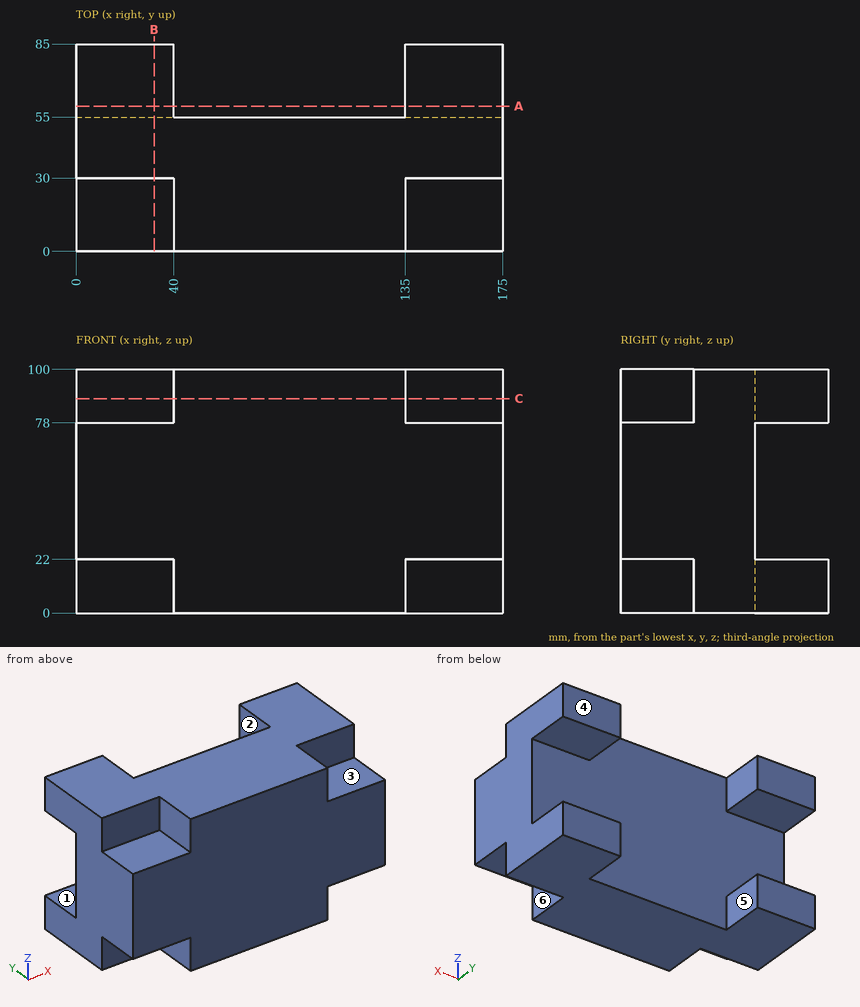
Verification items for this drawing (mm, ordinates from the low corner). A direction names the side the tool comes from. Give positions to 0.01 mm unless a question says otherwise; leave off trailing zeros. Loops run counter-clockwise (first coordinate to the right, second up) from the corner with the lowest first, then second, coordinate; pieces in that order, holes last.
1. Cross-section at C-C on z = 88. Record the cut outline in (x, y), and give its area (4 significant figures).
Derived:
outline: (0, 30) - (40, 30) - (40, 0) - (135, 0) - (135, 30) - (175, 30) - (175, 85) - (135, 85) - (135, 55) - (40, 55) - (40, 85) - (0, 85) - close
area: 9,625 mm2
2. Go/stop test with flat-tipped pins: P1, Ø17.5, axis at y = 17, z = 90.5, coming from the +X side; P2, Ø9, axis at x = 154, y = 12, coming from the +Z side; P3, Ø11, axis at x = 25.5, z = 90, coming from the -Y side. Record where each tip stops, or that it passes through.
Derived:
P1: stops at x = 135
P2: stops at z = 78
P3: stops at y = 30
3. Material ranges on probe 1 along Z at (x, y) = (140, 68.5); probe 2 along X at (y, z) = (58, 81.5); probe 3 along Y at (x, z) = (75, 18.5), recorded low to high.
Derived:
probe 1: z = 0 to 22, 78 to 100
probe 2: x = 0 to 40, 135 to 175
probe 3: y = 0 to 55
4. Cross-section at A-A on y = 59.5. Record the cut outline in (x, z).
Derived:
outline: (0, 0) - (40, 0) - (40, 22) - (0, 22) - close; (0, 78) - (40, 78) - (40, 100) - (0, 100) - close; (135, 0) - (175, 0) - (175, 22) - (135, 22) - close; (135, 78) - (175, 78) - (175, 100) - (135, 100) - close
5. Release check for a two-part mould opening along X. For the marked faces 4, 5 and 6 record: +X half, -X half, draft (parallel to the pull), parting line (faces both ways), or undercut.
Derived:
face 4: draft
face 5: undercut
face 6: +X half
6. Cross-section at B-B on x = 32. Record the cut outline in (y, z), and give its area (3 significant figures).
Derived:
outline: (0, 22) - (30, 22) - (30, 0) - (85, 0) - (85, 22) - (55, 22) - (55, 78) - (85, 78) - (85, 100) - (30, 100) - (30, 78) - (0, 78) - close
area: 5,500 mm2
7. Tool access check on the marked faces 1, 2 and 3. Record the directions out of +Z, -Z, +X, -X, +Y, -Y that give a thin tool (end or side, any length) a straight path to the whole face; none if there is none.
Derived:
face 1: +X, -X, +Y
face 2: +Z, -Z, +Y
face 3: +Z, +X, -Y
